Work out the finished part from the listing and answer in its coordinate system (mm). Coordinates: 2 decimals unless noted, no trailing zeros. Order: outer loops, then holes, each group sorted by start corner. A loop starts at its lowest first (then second) coordinate and runs counter-clockwise, first axis right, second up. Notation, with made-up numbers: (35, 31) - (81, 31) arc R28 ccw to (81, 56) - close; hole circle Ø6 at (17, 49). An arc over 180 degrees is marked (long way). Answer as a JSON object with one key per item and string values. Group by question number.
1) Find the intervals of material crossed by line 1 along Y through (x, z) = (0, 10.75); line 2 along X through (y, z) = (-6.75, 16.75), in increasing order.
2) Each of these flat-tipped pins is pushed along its axis until it touches: P1, Ø2, axis at x = -7.5, z = 18.5, coming from the +Y side; P2, Ø8, axis at y = 3.5, z = 16, coming from the -X side; P3, Ø5, axis at x = -5.5, z = 8, coming from the +Y side; P4, Ø4, axis at x = 3, z = 12.5, coming from the -Y side. Where does it stop, or does it pass through?
3) The mould has two halves that part along X. Classify faces 1 (the face through (-2.38, -10.74, 10.61)), 2 (the face through (5, 8, 0)), 3 (the face through (8.155, 2.568, 10.606)): released by +X, released by -X, zero draft, split by the parting line, or undercut.
4) Section A-A (y = 0) is taken. Give the vertices of the cut face in (x, z).
5) Section C-C (z = 19.5) is taken. Give the vertices of the cut face in (x, y), plus the area to 3 significant figures.
from build123d import *

# Parameters (mm, degrees)
SKETCH_1_R      = 11
SKETCH_1_R_2    = 8.55
EXTRUDE_1_DEPTH = 21.5
CHAMFER_1_SIZE  = 0.5


with BuildPart() as part:
    # 草图1 → 凸台-拉伸1 (new body)
    with BuildSketch(Plane.XY):
        Circle(SKETCH_1_R)
        Circle(SKETCH_1_R_2, mode=Mode.SUBTRACT)
    extrude(amount=EXTRUDE_1_DEPTH)

    # 倒角1
    chamfer_1_edges = [part.edges().sort_by_distance(p)[0] for p in [
        (-11, 0, 0),
        (-11, 0, 21.5),
        (-8.55, 0, 0),
        (-8.55, 0, 21.5),
    ]]
    chamfer(chamfer_1_edges, length=CHAMFER_1_SIZE)


solid = part.part
Report:
{
 "1": {"line 1": "y = -11 to -8.55, 8.55 to 11", "line 2": "x = -8.69 to -5.25, 5.25 to 8.69"},
 "2": {"P1": "stops at y = 8.87", "P2": "stops at x = -11", "P3": "stops at y = 10.58", "P4": "stops at y = -10.95"},
 "3": {"face 1": "split by the parting line", "face 2": "zero draft", "face 3": "undercut"},
 "4": {"outline": "(-11, 0.5) - (-10.5, 0) - (-9.05, 0) - (-8.55, 0.5) - (-8.55, 21) - (-9.05, 21.5) - (-10.5, 21.5) - (-11, 21) - close; (8.55, 0.5) - (9.05, 0) - (10.5, 0) - (11, 0.5) - (11, 21) - (10.5, 21.5) - (9.05, 21.5) - (8.55, 21) - close"},
 "5": {"outline": "circle Ø22 at (0, 0); hole circle Ø17.1 at (0, 0)", "area": "150 mm²"}
}
